The figure shows three views and two pictorial views of one solid part (mm, origin at its lowest corner). Answer the questions. A direction names the side the tool comes from. Coordinates: 2 decimals unless noted, no trailing zeros. Order: outer loops, then holes, each group sorted by start corner. A loop starts at its lowest first (then second) coordinate and runs counter-clockwise, first axis right, second up. Notation, with made-up numbers: (-3, 28) -> (36, 28) arc R27 ccw to (36, 66) -> close; hole circle Ø4 at (6.25, 46). An arc over 180 degrees is marked (long way). Return JSON: item names as keys, results as strings.
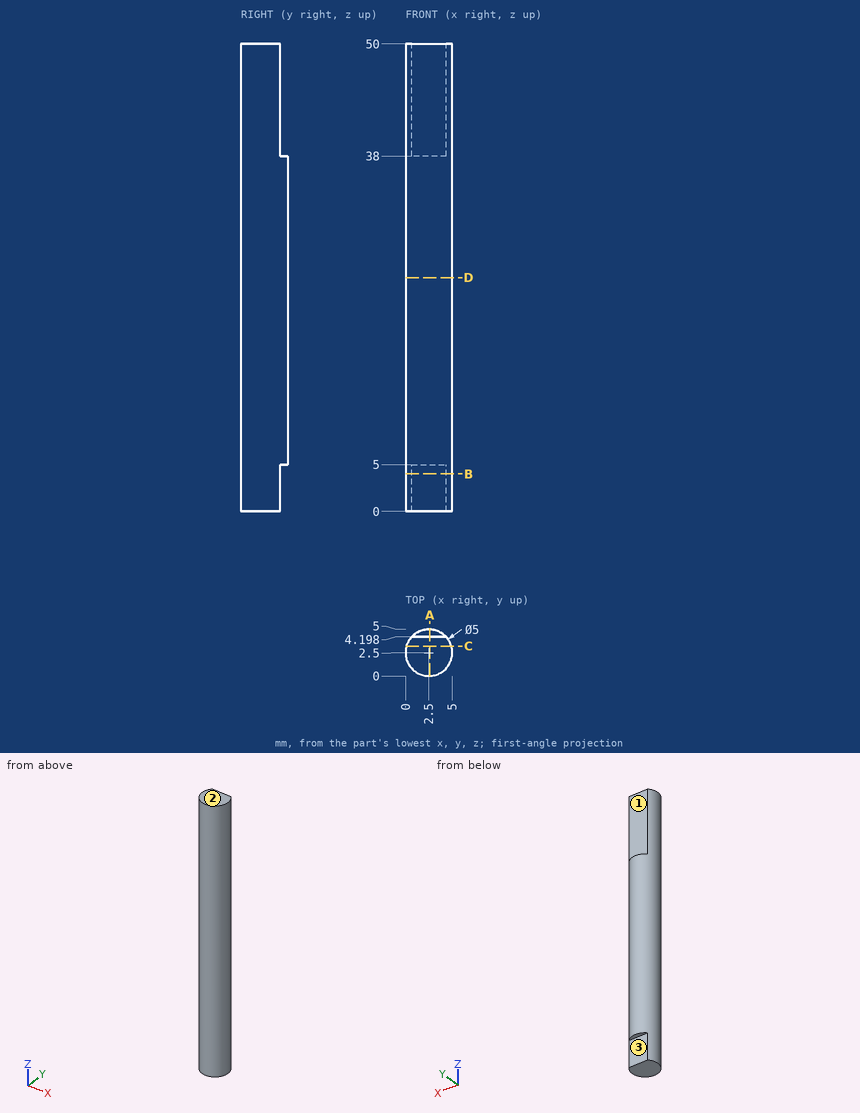
1. Each of these flat-tipped pins is pushed along its axis until it touches: pin 1 Ø1.8 at (x, z) = (2.5, 43) entering from +Y; pin 2 Ø1 at (y, z) = (3.5, 44.5) entering from +X. Where does it stop, or does it pass through?
Answer block:
{"pin 1": "stops at y = 4.2", "pin 2": "stops at x = 4.95"}
2. Consider line 1 (Y direction, x = 2.85, z = 27); line 2 (X direction, y = 0.9, z = 46); line 3 (X direction, y = 3.6, z = 26) (1 decimal). Determine where each line is inside the solid, lowest interval first. Write a range as from..to.
Answer block:
{"line 1": "y = 0.02..4.98", "line 2": "x = 0.58..4.42", "line 3": "x = 0.3..4.7"}
3. The part is cut by section C-C on y = 3.2. Give the vertices of the cut face in (x, z), and give its area (3 significant figures).
Answer block:
{"outline": "(0.1, 0) -> (4.9, 0) -> (4.9, 50) -> (0.1, 50) -> close", "area": "240 mm2"}
4. For the marked faces 1, 2 and 3, determine the directions among +Z, -Z, +X, -X, +Y, -Y from which every point of the face is accessible in a straight line to the end or side of a thin tool.
Answer block:
{"face 1": "+Z, +X, -X, +Y", "face 2": "+Z, +X, -X, +Y, -Y", "face 3": "-Z, +X, -X, +Y"}
5. The part is cut by section A-A on x = 2.6. Give the vertices of the cut face in (y, z).
Answer block:
{"outline": "(0, 0) -> (4.2, 0) -> (4.2, 5) -> (5, 5) -> (5, 38) -> (4.2, 38) -> (4.2, 50) -> (0, 50) -> close"}
6. The part is cut by section B-B on z = 4. Give the vertices of the cut face in (x, y) (3 decimals).
Answer block:
{"outline": "(0.665, 4.198) arc R2.5 ccw (long way) to (4.335, 4.198) -> close"}
7. The part is cut by section D-D on z = 25. Give the vertices of the cut face in (x, y), and give its area (3 significant figures).
Answer block:
{"outline": "circle Ø5 at (2.5, 2.5)", "area": "19.6 mm2"}
